Check sheet for the modelled part. Datum: model origin and axes. Units: mm. Face numbers are marked on the shaded views. Coordinates: 2 decimals unless noted, no trailing zeros. Loops run counter-clockwise (first coordinate to the right, second up) from the corner with the lowest first, then second, coordinate; pieces in that order, holes last. Notation, with made-up numbers: (41, -31.5) -> (71, -31.5) arc R23 ccw to (71, 5.5) -> close; hole circle Ø5 at (68, 77.25). An arc over 180 degrees is marked (long way). Use one line per item in the form item = value.
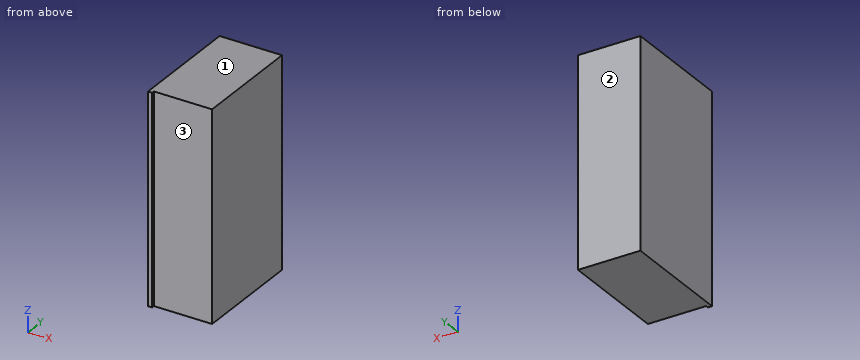
from build123d import *

# Parameters (mm, degrees)
EXTRUDE_1_DEPTH = 75


with BuildPart() as part:
    # 草图1 → 凸台-拉伸1 (new, symmetric)
    with BuildSketch(Plane.XY):
        Polygon((0, 0), (0, 82), (45, 82), (45, 2), (3, 2), (3, 0), align=None)
    extrude(amount=EXTRUDE_1_DEPTH, both=True)


solid = part.part
(1) Mould release check, pull along Y, two halves, no side actions. Record for the marked faces 1, 2 and 3: +Y half, -Y half, draft (parallel to the pull), parting line (faces both ways), or undercut.
Established:
face_1 = draft
face_2 = +Y half
face_3 = -Y half
(2) Scan line: line 1 along Y through (x, z) = (34, 33.5). Record every from-to range of solid material in increasing order.
Established:
line_1 = 2 to 82
(3) Section check B-B, the plane x = 22. Record the boundary of the cut face in (y, z).
Established:
outline = (2, -75) -> (82, -75) -> (82, 75) -> (2, 75) -> close
(4) Section check A-A, the plane z = 59. Record the boundary of the cut face in (x, y).
Established:
outline = (0, 0) -> (3, 0) -> (3, 2) -> (45, 2) -> (45, 82) -> (0, 82) -> close
(5) Go/stop test with flat-tipped pins: P1, Ø4, axis at x = 6.5, z = -17.5, coming from the -Y side; P2, Ø0.6, axis at y = 1, z = -24.5, coming from the +X side; P3, Ø8, axis at y = 47, z = -0.5, coming from the -X side. Record where each tip stops, or that it passes through.
Established:
P1 = 2
P2 = 3
P3 = 0
